The figure shows three views and two pictorial views of one solid part (mm, origin at its lowest corner). Answer the questions. A direction names the side the tool comes from. Give positions to 0.01 mm unless a question says otherwise; leave off trailing zeros. Order: outer loops, then holes, each group sorted by start corner. A loop starts at its lowest first (then second) coordinate and runs counter-clockwise, first axis right, second up. Notation, with made-up numbers: (61, 18.25) - (68, 18.25) arc R19 ccw to (68, 43.25) - close; hole circle Ø9 at (8, 48.25). An arc over 180 degrees is marked (long way). Use a Markdown table: item, result. Add a question column.
1. A cutting plane is placed at D-D on y = 16. Determine the outline of the cut face in (x, z).
2. Consider L1, parallel to X at y = 11, z = 14 (1 decimal); L2, parallel to Y at x = 8.5, z = 20.75; L3, parallel to X at y = 38.5, z = 21.5 (1 decimal). Determine where each line is inside the solid, lowest interval first.
3. Flat-ended cylindrical pins translate along their axes: P1, Ø10, axis at x = 5.5, z = 19, coming from the +Y side; P2, Ø3, axis at y = 36, z = 18.5, coming from the +X side; P3, Ø4, axis at y = 24.5, z = 8.5, coming from the +X side. Find the tip coordinate at first contact, or state that the pin passes through.
4. Which of the six approach directions +Z, -Z, +X, -X, +Y, -Y give full straight-line access (tool end or side, diameter ignored) to the marked faces 5, 6 and 7?
5. A cutting plane is placed at A-A on y = 6.5. Determine the outline of the cut face in (x, z).
6. For a pull along X with two mould halves and no side action, classify the marked faces 1, 2, 3 and 4 as released by +X, released by -X, zero draft, split by the parting line, or undercut.
7. A cutting plane is placed at C-C on x = 9. Determine the outline of the cut face in (y, z), and give its area (3 significant figures).
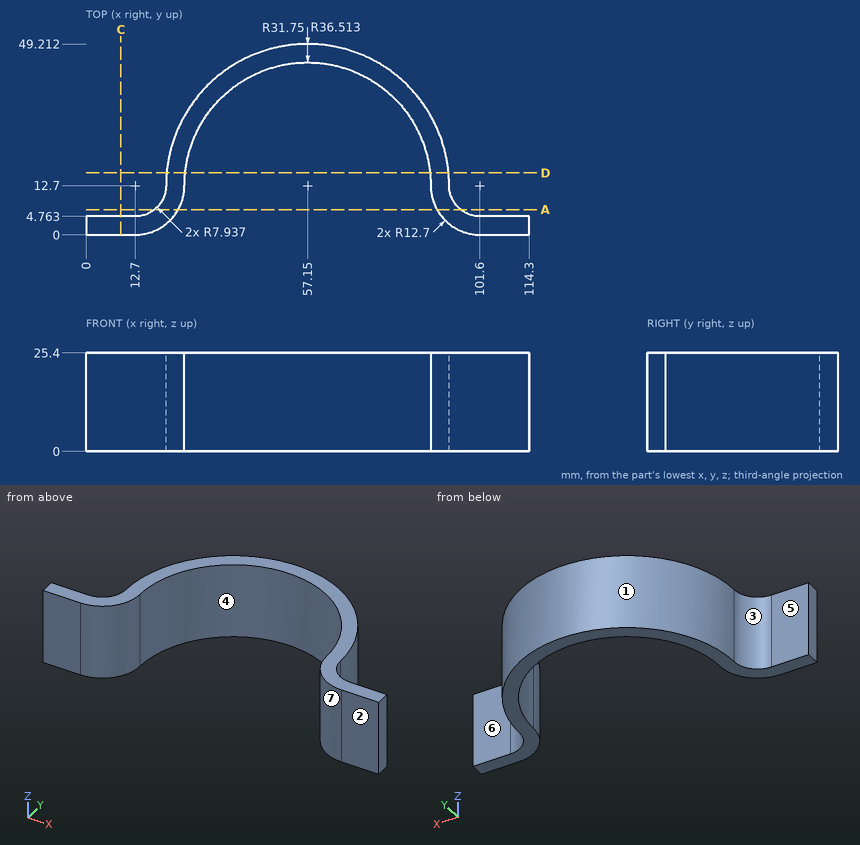
Output values:
| question | item | result |
|---|---|---|
| 1 | outline | (20.79, 0) - (25.57, 0) - (25.57, 25.4) - (20.79, 25.4) - close; (88.73, 0) - (93.51, 0) - (93.51, 25.4) - (88.73, 25.4) - close |
| 2 | L1 | 20.5 to 25.3, 89 to 93.8 |
| 2 | L2 | 0 to 4.76 |
| 2 | L3 | 31.3 to 38.6, 75.7 to 83 |
| 3 | P1 | y = 4.76 |
| 3 | P2 | x = 86.44 |
| 3 | P3 | x = 92.32 |
| 4 | face 5 | +Z, -Z, -X, +Y |
| 4 | face 6 | +Z, -Z, +X, +Y |
| 4 | face 7 | +Z, -Z, -Y |
| 5 | outline | (17.66, 0) - (23.78, 0) - (23.78, 25.4) - (17.66, 25.4) - close; (90.52, 0) - (96.64, 0) - (96.64, 25.4) - (90.52, 25.4) - close |
| 6 | face 1 | split by the parting line |
| 6 | face 2 | zero draft |
| 6 | face 3 | released by -X |
| 6 | face 4 | undercut |
| 7 | outline | (0, 0) - (4.76, 0) - (4.76, 25.4) - (0, 25.4) - close |
| 7 | area | 121 mm² |
